```python
from build123d import *

# Parameters (mm, degrees)
EDGE_FILLET_R0_2_R = 0.2


with BuildPart() as part:
    # Plug Profile Sketch → Plug Body Revolve (revolve)
    with BuildSketch(Plane.XY, mode=Mode.PRIVATE) as plug_body_revolve_sk:
        Polygon((0, 0), (-35, 0), (-35, 4), (-15, 4), (-15, 3), (-14, 3), (-14, 1.7), (-8.5, 1.7), (-8.5, 1.6), (-7.8, 1.6), (-7.8, 1.7), (-5.3, 1.7), (-5.3, 1.6), (-4.6, 1.6), (-4.6, 1.7), (-4.4, 1.7), (-4, 1.25), (-1.1, 1.6), (0, 0.5), align=None)
    revolve(plug_body_revolve_sk.sketch.rotate(Axis((0, 0, 0), (-1, 0, 0)), 90), axis=Axis((0, 0, 0), (-1, 0, 0)))

    # Edge Fillet R0.2
    edge_fillet_r0_2_edges = [part.edges().sort_by_distance(p)[0] for p in [
        (-1.1, 0, 1.6),
    ]]
    fillet(edge_fillet_r0_2_edges, radius=EDGE_FILLET_R0_2_R)


solid = part.part
```
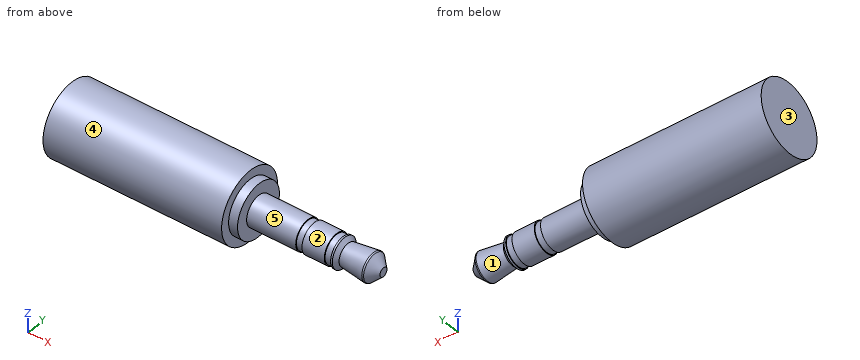
Input: part model. Units: mm. Frame: model coordinates. Face numbers are marked on the shaded views. A direction names the side the tool comes from. Coordinates: 2 decimals unless noted, no trailing zeros. Loops run counter-clockwise (first coordinate to the right, second up) from the corner with the lowest first, then second, coordinate; pieces in that order, holes last. Notation, with made-up numbers: M -16,15 L 10,15 A31 cw 10,39 Z; hole C -27.5,-2 d5. An arc over 180 degrees is marked long. Use a Markdown table: item, result. Add a question column.
1) Section A-A, the plane z = -2.25. Return the cut outline in (x, y).
2) Set-up query: the marked faces 4 and 5. Return all of +Z, -Z, +X, -X, +Y, -Y with unobstructed straight access to the full face (end or side cutting, diameter ignored); none if empty.
3) Section B-B, the plane y = -2.5. Return the cut outline in (x, z), plus the area to 3 significant figures.
4) Section C-C, the plane x = -22. Return the cut outline in (y, z), plus the area to 3 significant figures.
5) Draft query along X for the marked faces 1, 2 and 3. Return one class per face: +X half, -X half, draft (parallel to the pull), parting line (faces both ways), or undercut.
6) Line query: L1, parallel to X at y = 3.5, z = -1.5; L2, parallel to X at y = 2.5, z = -1; L3, parallel to Y at x = -27.5, z = -0.5. Output: solid intervals per line, ascending. Write a range as from..to.
7) Pin query (flat end, axial travel): P1, Ø1, axis at x = -21, z = 2, coming from the +Y side; P2, Ø2, axis at y = -2.5, z = -2.5, coming from the +X side; P3, Ø3, axis at x = -20.5, y = -2, coming from the -Z side. Return the tip coordinate at first contact, or that it passes through.
Answer below:
| question | item | result |
|---|---|---|
| 1 | outline | M -35,-3.31 L -15,-3.31 L -15,-1.98 L -14,-1.98 L -14,1.98 L -15,1.98 L -15,3.31 L -35,3.31 Z |
| 2 | face 4 | +X, -X |
| 2 | face 5 | +X |
| 3 | outline | M -35,-3.12 L -15,-3.12 L -15,-1.66 L -14,-1.66 L -14,1.66 L -15,1.66 L -15,3.12 L -35,3.12 Z |
| 3 | area | 128 mm2 |
| 4 | outline | C 0,0 d8 |
| 4 | area | 50.3 mm2 |
| 5 | face 1 | undercut |
| 5 | face 2 | draft |
| 5 | face 3 | -X half |
| 6 | L1 | -35..-15 |
| 6 | L2 | -35..-14 |
| 6 | L3 | -3.97..3.97 |
| 7 | P1 | y = 3.71 |
| 7 | P2 | x = -14 |
| 7 | P3 | z = -3.97 |
